from build123d import *

# Parameters (mm, degrees)
SKETCH1_R           = 85
BOSS_EXTRUDE1_DEPTH = 14
SKETCH2_R           = 55
SKETCH2_R_2         = 49
BOSS_EXTRUDE2_DEPTH = 14
FILLET1_R           = 5
FILLET2_R           = 1
CHAMFER1_SIZE       = 2
CHAMFER1_SIZE2      = 1.154700538
CHAMFER2_SIZE       = 1
CHAMFER2_SIZE2      = 0.577350269
BOSS_EXTRUDE3_DEPTH = 36
SKETCH5_R           = 6.75
CUT_EXTRUDE1_DEPTH  = 126.483066587
CIRPATTERN1_COUNT   = 6
M12_TAPPED_HOLE1_D  = 10.2


with BuildPart() as part:
    # Sketch1 → Boss-Extrude1 (new body)
    with BuildSketch(Plane(origin=(0, 0, 0), x_dir=(1, 0, 0), z_dir=(0, 1, 0))):
        with Locations(Location((0, 0, 0), (0, 0, 270))):
            Circle(SKETCH1_R)
    extrude(amount=BOSS_EXTRUDE1_DEPTH)

    # Sketch2 → Boss-Extrude2 (add)
    with BuildSketch(Plane(origin=(0, 14, 0), x_dir=(1, 0, 0), z_dir=(0, 1, 0))):
        with Locations(Location((0, 0, 0), (0, 0, 270))):
            Circle(SKETCH2_R)
        with Locations(Location((0, 0, 0), (0, 0, 270))):
            Circle(SKETCH2_R_2, mode=Mode.SUBTRACT)
    extrude(amount=BOSS_EXTRUDE2_DEPTH)

    # Fillet1
    fillet1_edges = [part.edges().sort_by_distance(p)[0] for p in [
        (0, 14, -49),
    ]]
    fillet(fillet1_edges, radius=FILLET1_R)

    # Fillet2
    fillet2_edges = [part.edges().sort_by_distance(p)[0] for p in [
        (0, 14, -55),
    ]]
    fillet(fillet2_edges, radius=FILLET2_R)

    # Chamfer1
    chamfer1_edges = [part.edges().sort_by_distance(p)[0] for p in [
        (0, 0, -85),
    ]]
    chamfer1_side = [part.faces().sort_by_distance(p)[0] for p in [
        (0, 0, 0),
    ]]
    chamfer(chamfer1_edges, length=CHAMFER1_SIZE, length2=CHAMFER1_SIZE2, reference=chamfer1_side[0])

    # Chamfer2
    chamfer2_edges = [part.edges().sort_by_distance(p)[0] for p in [
        (0, 28, -55),
    ]]
    chamfer2_side = [part.faces().sort_by_distance(p)[0] for p in [
        (0, 21.5, -55),
    ]]
    chamfer(chamfer2_edges, length=CHAMFER2_SIZE, length2=CHAMFER2_SIZE2, reference=chamfer2_side[0])

    # Sketch3 → Boss-Extrude3 (add)
    with BuildSketch(Plane.XZ):
        with BuildLine():
            Line((-53, 0), (-50, 0))
            ThreePointArc((-50, 0), (0, 50), (50, 0))
            Line((50, 0), (53, 0))
            ThreePointArc((53, 0), (0, 53), (-53, 0))
        make_face()
    extrude(amount=BOSS_EXTRUDE3_DEPTH)

    # Sketch4 → Cut-Revolve1 (revolve, cut)
    with BuildSketch(Plane.XY):
        Polygon((-46, 10.5), (-46, 3.5), (-38.5, 2.579115793), (-38.5, 0), (0, 0), (0, 14), (-38.5, 14), (-38.5, 11.420884207), align=None)
    revolve(axis=Axis((0, 14, 0), (0, -1, 0)), mode=Mode.SUBTRACT)

    # Sketch5 → Cut-Extrude1 (cut, through all)
    with BuildSketch(Plane.XZ):
        with Locations(Location((-35, 60.621778265, 0), (0, 0, 270))):
            Circle(SKETCH5_R)
    cut_extrude1 = extrude(amount=-CUT_EXTRUDE1_DEPTH, mode=Mode.SUBTRACT)

    # CirPattern1: Cut-Extrude1 ×6 about axis
    cirpattern1_axis = Axis((0, 0, 0), (0, 1, 0))
    for i in range(1, CIRPATTERN1_COUNT):
        add(cut_extrude1.rotate(cirpattern1_axis, i * 360 / CIRPATTERN1_COUNT), mode=Mode.SUBTRACT)

    # M12 Tapped Hole1 (through all)
    with Locations(Plane(origin=(0, 0, 0), x_dir=(-1, 0, 0), z_dir=(0, -1, 0))):
        with Locations((-60.621778265, -35), (60.621778265, 35)):
            Hole(M12_TAPPED_HOLE1_D / 2)


solid = part.part
Work out the finished part from the listing and answer in its coordinate system (mm). A direction names the side the tool comes from. Round coordinates to 2 decimals unless told otherwise and drop trailing zeros. Write each loop counter-clockwise with the first axis right and the second up, starting at its lowest first coordinate (ties: lowest second). Pieces come first, ordered by that corner, then holes. Notation, with made-up numbers: M 61.5,-32.75 L 84.5,-32.75 A23 cw 84.5,-15.75 Z; hole C 29,-31 d10. An arc over 180 degrees is marked long. Use a Markdown table: item, result.
1) Which of the six approach directions +Z, -Z, +X, -X, +Y, -Y give full straight-line access (tool end or side, diameter ignored) to faces 1 (the face through (30.55, 1.27, 23.43)), 2 (the face through (14.718, 23.437, 46.737)), 3 (the face through (5.059, 2.624, -38.533))?
Taken from the geometry:
| item | result |
|---|---|
| face 1 | +Y, -Y |
| face 2 | +Y |
| face 3 | none |
2) Determine the mould class of faces 4 (the face through (1.165, -17.748, 52.987)), 5 (the face through (76.693, 6.902, 0.879)), 6 (the face through (-55, 14, 18)) for opening direction X: pulls with the +X half, pulls with the -X half, needs draft (parallel to the pull), parting line crosses it, or undercut.
Taken from the geometry:
| item | result |
|---|---|
| face 4 | parting line crosses it |
| face 5 | undercut |
| face 6 | needs draft |
3) Flat-ended cylindrical pins translate along their axes: pin 1 (5 mm diameter, centred on x = 35, y = -3.5, fed in from -Z); pin 2 (1.5 mm diameter, centred on x = 51.5, y = -13, fed in from -Z); pin 3 (12 mm diameter, centred on y = -1, z = 52.5, fed in from -X). Find the tip coordinate at first contact, or state that the pin passes through.
Taken from the geometry:
| item | result |
|---|---|
| pin 1 | stops at z = 33.07 |
| pin 2 | stops at z = 0 |
| pin 3 | stops at x = -70.89 |
4) Consider line 1 (X direction, y = 13.1, z = 0); line 2 (X direction, y = 8, z = 0); line 3 (Z direction, x = -40, y = 9.5). Determine where each line is inside the solid, lowest interval first. Write a range as [from, to].
Taken from the geometry:
| item | result |
|---|---|
| line 1 | x = [-85, -76.75], [-63.25, -38.5], [38.5, 63.25], [76.75, 85] |
| line 2 | x = [-85, -76.75], [-63.25, -46], [46, 63.25], [76.75, 85] |
| line 3 | z = [-75, -65.16], [-56.09, -22.72], [22.72, 56.09], [65.16, 75] |
5) The part is cut by section D-D on y = -17. Give the vertices of the cut face in (x, z), plus the area to 3 significant figures.
Taken from the geometry:
| item | result |
|---|---|
| outline | M -53,0 L -50,0 A50 cw 50,0 L 53,0 A53 ccw Z |
| area | 485 mm2 |
6) The part is cut by section A-A on y = 5.5. State how many separate pieces and enclosed holes the cut face has, plus the area to 3 significant figures.
Taken from the geometry:
| item | result |
|---|---|
| separate pieces | 1 |
| enclosed holes | 9 |
| area | 15,000 mm2 |
